```python
from build123d import *

# Parameters (mm, degrees)
SKETCH_1_W                = 350
SKETCH_1_H                = 160
EXTRUDE_1_DEPTH           = 16
HOLE_WIZARD_M10_1_D       = 8.5
HOLE_WIZARD_10_5_10_5_1_D = 10.5
CHAMFER_1_SIZE            = 5


with BuildPart() as part:
    # 草图1 → 凸台-拉伸1 (new body)
    with BuildSketch(Plane(origin=(0, 0, 0), x_dir=(0, 0, -1), z_dir=(1, 0, 0))):
        Rectangle(SKETCH_1_W, SKETCH_1_H)
    extrude(amount=EXTRUDE_1_DEPTH)

    # M10 螺纹孔1 (through all)
    with Locations(Plane(origin=(16, 0, 0), x_dir=(0, 0, -1), z_dir=(1, 0, 0))):
        with Locations((-115, 50), (-115, -50), (105, 50), (105, -50), (-65, 50), (-65, -50)):
            Hole(HOLE_WIZARD_M10_1_D / 2)

    # Ø10.5 (10.5) 直径孔1 (through all)
    with Locations(Plane.ZY):
        with Locations((-160, 40), (-160, -40), (160, 40), (160, -40)):
            Hole(HOLE_WIZARD_10_5_10_5_1_D / 2)

    # 倒角1
    chamfer_1_edges = [part.edges().sort_by_distance(p)[0] for p in [
        (8, -80, -175),
        (8, -80, 175),
        (8, 80, 175),
        (8, 80, -175),
    ]]
    chamfer(chamfer_1_edges, length=CHAMFER_1_SIZE)


solid = part.part
```
Source: CAD feature listing. Evaluate the final solid. Frame: model axes, mm. Coordinates: 2 decimals unless noted, no trailing zeros. Order: outer loops, then holes, each group sorted by start corner. A loop starts at its lowest first (then second) coordinate and runs counter-clockwise, first axis right, second up. Notation, with made-up numbers: M 57.5,8.5 L 92.5,8.5 A17 ccw 92.5,19.5 Z; hole C -18,-3 d10. An arc over 180 degrees is marked long. Write each question's results on one line, items separated by ' | '. Start each with the question number.
1) Draft query along Y for faces 1 (the face through (16, 1, 2)), 2 (the face through (8, 80, 2)), 3 (the face through (7.888, -49.813, -109.246)). Return one class per face: released by +Y, released by -Y, zero draft, split by the parting line, or undercut.
2) Contact query for a flat-ended pin moving along its axis: pin 1 Ø6.5 at (y, z) = (-40, -160) entering from +X. Output: stop coordinate, or through.
3) Line query: line 1 (Y direction, x = 6.5, z = 65); line 2 (Y direction, x = 10.25, z = 160); line 3 (Z direction, x = 4, y = 52.5). Output: solid intervals per line, ascending. Write a range as from..to.
4) Section query B-B (z = 115). Return the cut outline in (x, y).
5) Section query A-A (z = -160). Return the cut outline in (x, y).
Answers:
1) face 1: zero draft | face 2: released by +Y | face 3: undercut
2) pin 1: passes through
3) line 1: y = -80..-54.25, -45.75..45.75, 54.25..80 | line 2: y = -80..-45.25, -34.75..34.75, 45.25..80 | line 3: z = -175..-108.44, -101.56..61.56, 68.44..111.56, 118.44..175
4) outline: M 0,-80 L 16,-80 L 16,-54.25 L 0,-54.25 Z; M 0,-45.75 L 16,-45.75 L 16,45.75 L 0,45.75 Z; M 0,54.25 L 16,54.25 L 16,80 L 0,80 Z
5) outline: M 0,-80 L 16,-80 L 16,-45.25 L 0,-45.25 Z; M 0,-34.75 L 16,-34.75 L 16,34.75 L 0,34.75 Z; M 0,45.25 L 16,45.25 L 16,80 L 0,80 Z
